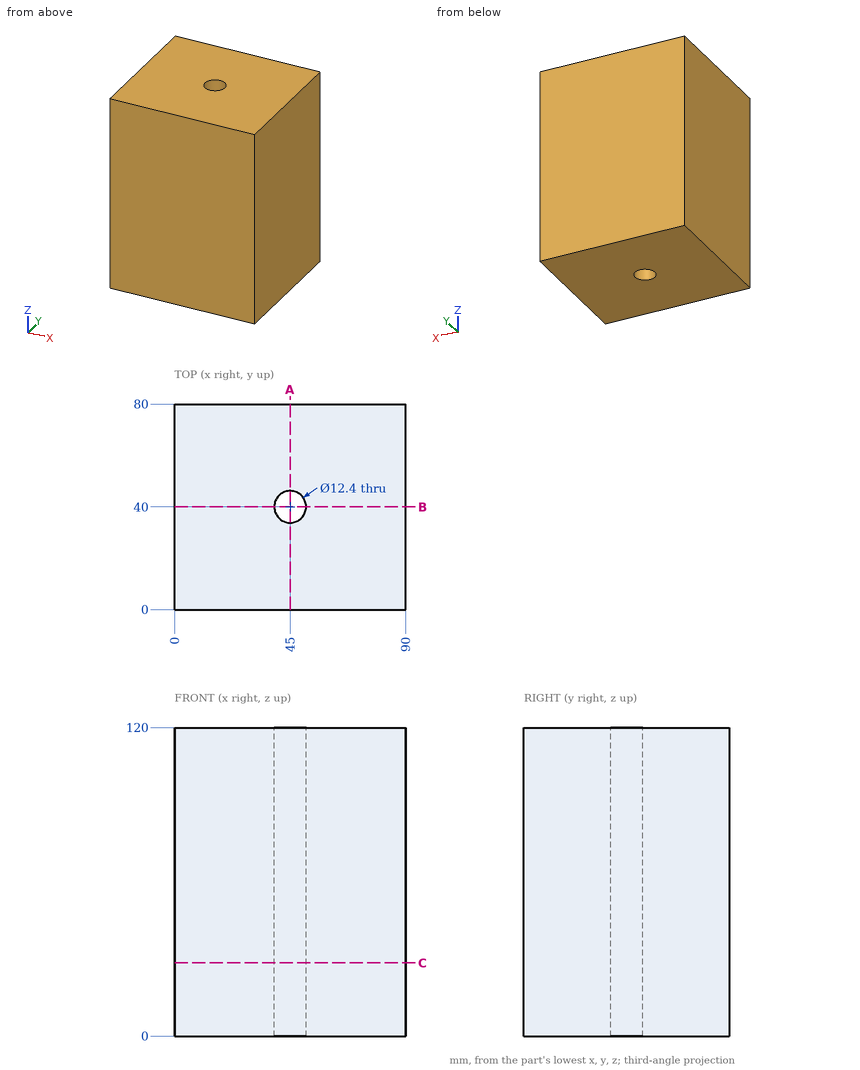
Geometry check sheet. Reference: drawing and pictorial views, mm from the part's lowest x, y, z. Give positions to 0.01 mm unless a question says otherwise; leave off trailing zeros. Order: outer loops, then holes, each group sorted by start corner. A loop starts at its lowest first (then second) coordinate and runs counter-clockwise, first axis right, second up. Notation, with made-up numbers: M 11,3.25 L 34,3.25 A29 ccw 34,29.25 Z; hole C -34,-22 d2. An arc over 180 degrees is marked long. Answer in a Markdown table with one row per item. Add a question column.
Item 1: Section check B-B, the plane y = 40. Enter the section's corners in (x, z), and give its area (3 significant figures).
Item 2: Scan lines: probe 1 along Y at (x, z) = (45, 71); probe 2 along X at (y, z) = (41, 29.5); probe 3 along X at (y, z) = (42.5, 63). Record each from-to range of solid material in increasing order. Write a range as from..to.
Item 3: Section check C-C, the plane z = 28.5. Enter the section's corners in (x, y).
Item 4: Section check A-A, the plane x = 45. Enter the section's corners in (y, z).
Item 5: Gauge pin test, flat ends, axial feed: pin 1 (3 mm diameter, centred on x = 11.5, y = 45, fed in from -Z); pin 2 (7.5 mm diameter, centred on x = 45, y = 40, fed in from -Z). Record the tip position at first contact, or that the pin passes through.
Filled sheet:
| question | item | result |
|---|---|---|
| 1 | outline | M 0,0 L 38.8,0 L 38.8,120 L 0,120 Z; M 51.2,0 L 90,0 L 90,120 L 51.2,120 Z |
| 1 | area | 9,310 mm^2 |
| 2 | probe 1 | y = 0..33.8, 46.2..80 |
| 2 | probe 2 | x = 0..38.88, 51.12..90 |
| 2 | probe 3 | x = 0..39.33, 50.67..90 |
| 3 | outline | M 0,0 L 90,0 L 90,80 L 0,80 Z; hole C 45,40 d12.4 |
| 4 | outline | M 0,0 L 33.8,0 L 33.8,120 L 0,120 Z; M 46.2,0 L 80,0 L 80,120 L 46.2,120 Z |
| 5 | pin 1 | stops at z = 0 |
| 5 | pin 2 | passes through |
